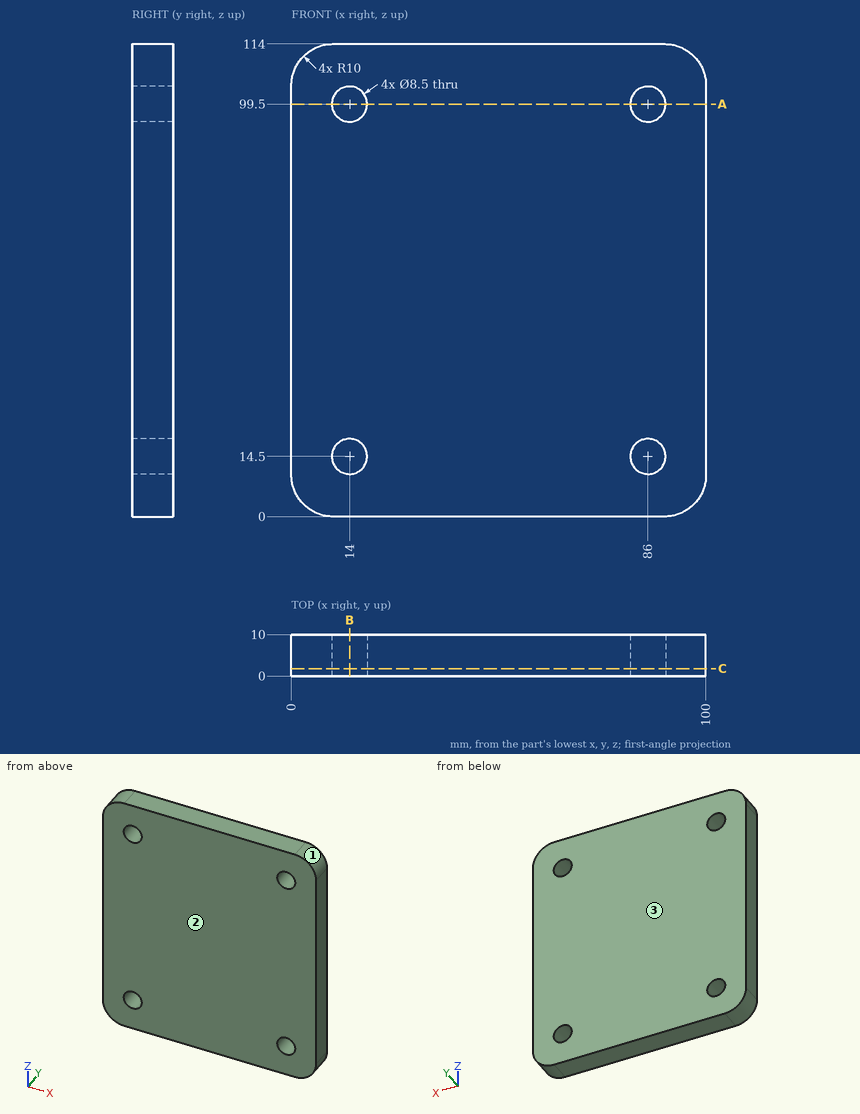
Here's the drawing with two shaded views (mm, measured from the low corner). I have some questions. Give positions to 0.01 mm unless a question says otherwise; leave off trailing zeros. Loops run counter-clockwise (first coordinate to the right, second up) from the corner with the lowest first, then second, coordinate; pieces in that order, holes last. Notation, with made-up numbers: (42, 61) - (74, 61) arc R20 ccw to (74, 73) - close; hole circle Ø8 at (56.25, -11.75). An arc over 180 degrees is marked (long way). Return JSON: item names as keys, results as strings.
1. I want a section at B-B on x = 14. Please give me the cut outline in (y, z).
Output values:
{"outline": "(0, 0) - (10, 0) - (10, 10.25) - (0, 10.25) - close; (0, 18.75) - (10, 18.75) - (10, 95.25) - (0, 95.25) - close; (0, 103.75) - (10, 103.75) - (10, 114) - (0, 114) - close"}
2. I want a section at C-C on y = 1.75. Please give me the cut outline in (x, z).
Output values:
{"outline": "(0, 10) arc R10 ccw to (10, 0) - (90, 0) arc R10 ccw to (100, 10) - (100, 104) arc R10 ccw to (90, 114) - (10, 114) arc R10 ccw to (0, 104) - close; hole circle Ø8.5 at (14, 14.5); hole circle Ø8.5 at (14, 99.5); hole circle Ø8.5 at (86, 14.5); hole circle Ø8.5 at (86, 99.5)"}
3. I'm going to push a flat-ended pin straight in: pin 1 Ø7 at (x, z) = (86, 14.5) entering from -Y. Where does the tip first touch, or does it pass through?
Output values:
{"pin 1": "passes through"}
4. We'd pull the mould along Y, two halves only. Please class the marked faces 1, 2 and 3: +Y half, -Y half, draft (parallel to the pull), parting line (faces both ways), or undercut.
Output values:
{"face 1": "draft", "face 2": "-Y half", "face 3": "+Y half"}
5. If I drill on line 1 (X direction, y = 7, z = 99.5); line 2 (Z direction, x = 14, y = 5.75); line 3 (X direction, y = 1.75, z = 96), over which ranges is the centre line in solid material (lowest first)?
Output values:
{"line 1": "x = 0 to 9.75, 18.25 to 81.75, 90.25 to 100", "line 2": "z = 0 to 10.25, 18.75 to 95.25, 103.75 to 114", "line 3": "x = 0 to 11.59, 16.41 to 83.59, 88.41 to 100"}
6. I want a section at A-A on z = 99.5. Please give me the cut outline in (x, y), and give its area (3 significant figures).
Output values:
{"outline": "(0, 0) - (9.75, 0) - (9.75, 10) - (0, 10) - close; (18.25, 0) - (81.75, 0) - (81.75, 10) - (18.25, 10) - close; (90.25, 0) - (100, 0) - (100, 10) - (90.25, 10) - close", "area": "830 mm²"}
